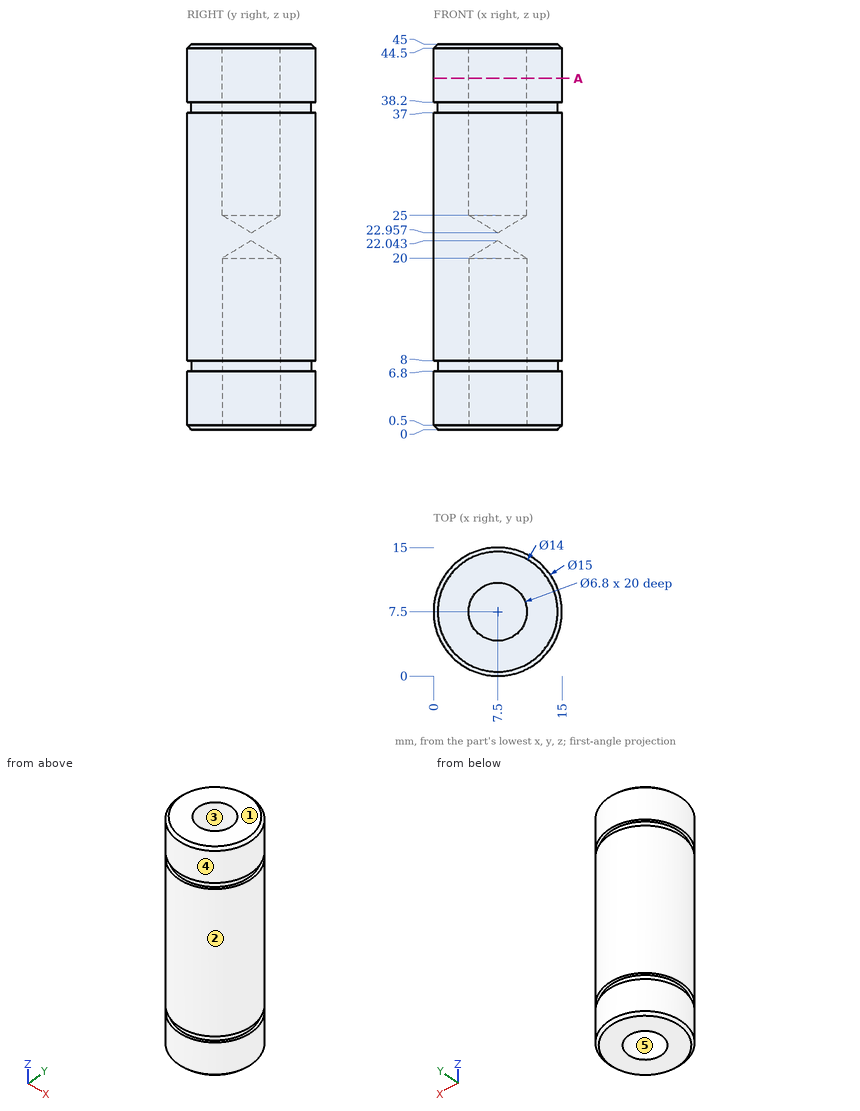
For this review, use the dimensioned drawing (mm, ordinates from the lowest corner) and the shaded views. A direction names the side the tool comes from. Coordinates: 2 decimals unless noted, no trailing zeros. Write each loop counter-clockwise with the first axis right and the second up, starting at its lowest first coordinate (ties: lowest second). Pieces come first, ordered by that corner, then holes. Notation, with made-up numbers: (21.5, 67.5) -> (61.5, 67.5) arc R28 cw to (61.5, 104.5) -> close; hole circle Ø3 at (-16, -18). An arc over 180 degrees is marked (long way). Write each question's results on one line, items separated by ' | '. Start each with the question number.
(1) Tool access review of the marked faces 4 and 5: name each direction out of +Z, -Z, +X, -X, +Y, -Y from which nothing blocks a thin tool from reaching the whole face with its end or side.
(2) The part is to be moulded in two halves that separate along X. For the marked faces 1, 2 and 3, say which applies: pulls with the +X half, pulls with the -X half, needs draft (parallel to the pull), parting line crosses it, or undercut.
(3) Take a section at A-A on z = 41. Write out the cut boundary in (x, y), and give its area (3 significant figures).
(4) For line 1 along Y through (x, z) = (7.5, 10); line 2 along X through (y, z) = (8, 23.5); line 3 along Y through (x, z) = (5.75, 31.5) (3 decimals), list the stretches that pass through material, from the lowest coordinate up. Write a range as from..to.
(5) Clearance check with flat-ended pins moving along their axes: P1, Ø1.5, axis at y = 10, z = 36.5, coming from the +X side; P2, Ø4, axis at x = 7.5, y = 7.5, coming from the -Z side; P3, Ø6, axis at x = 7.5, y = 7.5, coming from the -Z side. State where each tip first meets the part, or that it passes through.
Results found:
1) face 4: +Z, -Z | face 5: -Z
2) face 1: needs draft | face 2: parting line crosses it | face 3: undercut
3) outline: circle Ø15 at (7.5, 7.5); hole circle Ø6.8 at (7.5, 7.5) | area: 140 mm2
4) line 1: y = 0..4.1, 10.9..15 | line 2: x = 0.02..6.75, 8.25..14.98 | line 3: y = 0.207..4.585, 10.415..14.793
5) P1: stops at x = 14.79 | P2: stops at z = 20.84 | P3: stops at z = 20.24
